```python
from build123d import *

# Parameters (mm, degrees)
HUB_PROFILE_SKETCH_R           = 4.5
HUB_CYLINDER_DEPTH             = 6
ARM_START                      = -4
ARM_DEPTH                      = 3
FLAT_EAR_PROFILE_SKETCH_R      = 0.7
FLAT_MOUNTING_EAR_DEPTH        = 1.6
UPRIGHT_EAR_PROFILE_SKETCH_R   = 0.7
UPRIGHT_MOUNTING_EAR_DEPTH     = 0.8
UPRIGHT_EAR_EXTENSION_SKETCH_W = 1.6
UPRIGHT_EAR_EXTENSION_SKETCH_H = 3.2
UPRIGHT_EAR_EXTENSION_DEPTH    = 0.8
HUB_BORE_CBORE_4_4_D           = 4.4
HUB_BORE_CBORE_4_4_DEPTH       = 100
HUB_BORE_CBORE_4_4_CBORE_D     = 6.4
HUB_BORE_CBORE_4_4_CBORE_DEPTH = 2
ARM_FRAME_CUT_DEPTH            = 18.786996987
ARM_FRAME_CUT_DEPTH_BACK       = 18.786996987
ARM_FRAME_CUT_SKETCH_R         = 0.6
ARM_START_2                    = -1
ARM_WINDOW_CUT_A_DEPTH         = 1
ARM_START_3                    = -3
ARM_WINDOW_CUT_B_DEPTH         = 1


with BuildPart() as part:
    # Hub Profile Sketch → Hub Cylinder (new body)
    with BuildSketch(Plane(origin=(0, 0, 0), x_dir=(1, 0, 0), z_dir=(0, 1, 0))):
        with Locations(Location((0, 0, 0), (0, 0, 270))):
            Circle(HUB_PROFILE_SKETCH_R)
    extrude(amount=HUB_CYLINDER_DEPTH)

    # Arm Profile Sketch → Arm (add)
    with BuildSketch(Plane(origin=(0, 6, 0), x_dir=(1, 0, 0), z_dir=(0, 1, 0)).offset(ARM_START)):
        with BuildLine():
            Line((1.029929577, 4.380553055), (14.486091549, 1.216820293))
            ThreePointArc((14.486091549, 1.216820293), (15.45, 0), (14.486091549, -1.216820293))
            Line((14.486091549, -1.216820293), (1.029929577, -4.380553055))
            ThreePointArc((1.029929577, -4.380553055), (4.5, 0), (1.029929577, 4.380553055))
        make_face()
    extrude(amount=ARM_DEPTH)

    # Flat Ear Profile Sketch → Flat Mounting Ear (add)
    # profile 1 of 2: a face of its own
    with BuildSketch(Plane.XZ):
        with BuildLine():
            Line((-0.677946652, 4.448638931), (-1.807326015, 6.445430372))
            ThreePointArc((-1.807326015, 6.445430372), (-3.987692308, 7.050412049), (-4.592673985, 4.870045756))
            Line((-4.592673985, 4.870045756), (-3.463294622, 2.873254315))
            ThreePointArc((-3.463294622, 2.873254315), (-2.215384615, 3.916895583), (-0.677946652, 4.448638931))
        make_face()
        with Locations(Location((-3.2, 5.657738064, 0), (0, 0, 270))):
            Circle(FLAT_EAR_PROFILE_SKETCH_R, mode=Mode.SUBTRACT)
    # profile 2 of 2: a face of its own
    with BuildSketch(Plane.XZ):
        with BuildLine():
            Line((-0.677946652, -4.448638931), (-1.807326015, -6.445430372))
            ThreePointArc((-1.807326015, -6.445430372), (-3.987692308, -7.050412049), (-4.592673985, -4.870045756))
            Line((-4.592673985, -4.870045756), (-3.463294622, -2.873254315))
            ThreePointArc((-3.463294622, -2.873254315), (-2.215384615, -3.916895583), (-0.677946652, -4.448638931))
        make_face()
        with Locations(Location((-3.2, -5.657738064, 0), (0, 0, 270))):
            Circle(FLAT_EAR_PROFILE_SKETCH_R, mode=Mode.SUBTRACT)
    extrude(amount=-FLAT_MOUNTING_EAR_DEPTH)



with BuildPart() as body_2:
    # Upright Ear Profile Sketch → Upright Mounting Ear (new, symmetric)
    with BuildSketch(Plane.XY):
        with BuildLine():
            Line((-4.5, 6), (-6.5, 6))
            ThreePointArc((-6.5, 6), (-8.1, 4.4), (-6.5, 2.8))
            Line((-6.5, 2.8), (-4.5, 2.8))
            Line((-4.5, 2.8), (-4.5, 6))
        make_face()
        with Locations((-6.5, 4.4)):
            Circle(UPRIGHT_EAR_PROFILE_SKETCH_R, mode=Mode.SUBTRACT)
    extrude(amount=UPRIGHT_MOUNTING_EAR_DEPTH, both=True)


with BuildPart() as part_1:
    add(part.part)

    add(body_2.part)  # Upright Ear Extension merges body 2
    # Upright Ear Extension Sketch → Upright Ear Extension (add, symmetric)
    with BuildSketch(Plane(origin=(-4.5, 0, 0), x_dir=(0, 0, -1), z_dir=(1, 0, 0))):
        with Locations((0, 4.4)):
            Rectangle(UPRIGHT_EAR_EXTENSION_SKETCH_W, UPRIGHT_EAR_EXTENSION_SKETCH_H)
    extrude(amount=UPRIGHT_EAR_EXTENSION_DEPTH, both=True)

    # Hub Bore CBore _4.4
    with Locations(Plane(origin=(0, 6, 0), x_dir=(1, 0, 0), z_dir=(0, 1, 0))):
        with Locations((0, 0)):
            CounterBoreHole(HUB_BORE_CBORE_4_4_D / 2, HUB_BORE_CBORE_4_4_CBORE_D / 2, HUB_BORE_CBORE_4_4_CBORE_DEPTH, depth=HUB_BORE_CBORE_4_4_DEPTH)

    # Arm Frame Cut Sketch → Arm Frame Cut (cut, two sides: drawn at the far end of the back side and taken through both)
    with BuildSketch(Plane(origin=(0, 5, 0), x_dir=(1, 0, 0), z_dir=(0, 1, 0)).offset(-ARM_FRAME_CUT_DEPTH_BACK)):
        with Locations(Location((14.2, 0, 0), (0, 0, 270))):
            Circle(ARM_FRAME_CUT_SKETCH_R)
        with BuildLine():
            Line((12.018798086, 0.769648107), (5.510009379, 2.299955792))
            ThreePointArc((5.510009379, 2.299955792), (5.216619254, 2.20665809), (5.159898403, 1.904061046))
            ThreePointArc((5.159898403, 1.904061046), (5.5, 0), (5.159898403, -1.904061046))
            ThreePointArc((5.159898403, -1.904061046), (5.216619254, -2.20665809), (5.510009379, -2.299955792))
            Line((5.510009379, -2.299955792), (12.018798086, -0.769648107))
            ThreePointArc((12.018798086, -0.769648107), (12.203456694, -0.638324285), (12.243596621, -0.415314119))
            ThreePointArc((12.243596621, -0.415314119), (12.2, 0), (12.243596621, 0.415314119))
            ThreePointArc((12.243596621, 0.415314119), (12.203456694, 0.638324285), (12.018798086, 0.769648107))
        make_face()
    extrude(amount=ARM_FRAME_CUT_DEPTH + ARM_FRAME_CUT_DEPTH_BACK, mode=Mode.SUBTRACT)

    # Arm Window Sketch → Arm Window Cut A (cut)
    with BuildSketch(Plane(origin=(0, 5, 0), x_dir=(1, 0, 0), z_dir=(0, 1, 0)).offset(ARM_START_2)):
        with BuildLine():
            Line((12.96628349, 1.574148524), (4.108268481, 3.656792323))
            ThreePointArc((4.108268481, 3.656792323), (4.716221589, 2.829709158), (5.159898403, 1.904061046))
            ThreePointArc((5.159898403, 1.904061046), (5.216619254, 2.20665809), (5.510009379, 2.299955792))
            Line((5.510009379, 2.299955792), (12.018798086, 0.769648107))
            ThreePointArc((12.018798086, 0.769648107), (12.203456694, 0.638324285), (12.243596621, 0.415314119))
            ThreePointArc((12.243596621, 0.415314119), (12.502961249, 1.058328625), (12.96628349, 1.574148524))
        make_face()
    extrude(amount=ARM_WINDOW_CUT_A_DEPTH, mode=Mode.SUBTRACT)

    # Sketch12_2 → Arm Window Cut B (cut)
    with BuildSketch(Plane(origin=(0, 5, 0), x_dir=(1, 0, 0), z_dir=(0, 1, 0)).offset(ARM_START_3)):
        with BuildLine():
            Line((12.96628349, 1.574148524), (4.108268481, 3.656792323))
            ThreePointArc((4.108268481, 3.656792323), (4.716221589, 2.829709158), (5.159898403, 1.904061046))
            ThreePointArc((5.159898403, 1.904061046), (5.216619254, 2.20665809), (5.510009379, 2.299955792))
            Line((5.510009379, 2.299955792), (12.018798086, 0.769648107))
            ThreePointArc((12.018798086, 0.769648107), (12.203456694, 0.638324285), (12.243596621, 0.415314119))
            ThreePointArc((12.243596621, 0.415314119), (12.502961249, 1.058328625), (12.96628349, 1.574148524))
        make_face()
    extrude(amount=ARM_WINDOW_CUT_B_DEPTH, mode=Mode.SUBTRACT)


solid = part_1.part
```
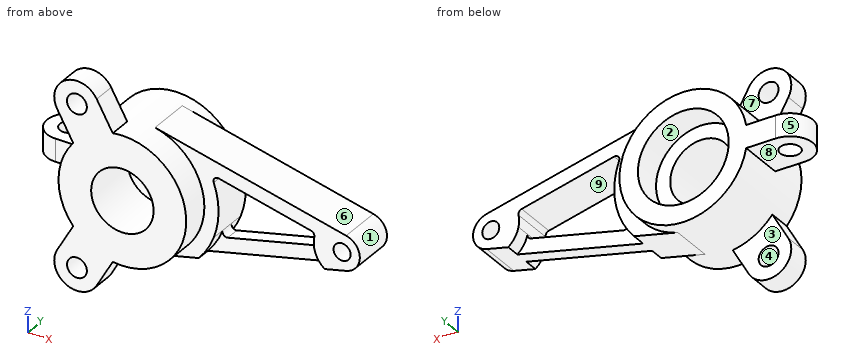
Check sheet for the modelled part. Datum: model origin and axes. Units: mm. Face numbers are marked on the shaded views. A direction names the side the tool comes from. Coordinates: 2 decimals unless noted, no trailing zeros. Order: outer loops, then holes, each group sorted by start corner. A loop starts at its lowest first (then second) coordinate and runs counter-clockwise, first axis right, second up. Notation, with made-up numbers: M -18.5,-22 L 13.5,-22 A34 cw 13.5,13 Z; hole C 16.25,48.25 d3. An arc over 180 degrees is marked long. One line per question, with ' | ' between items. Start each with the question number.
Item 1: Sectioned sample at A-A on z = 0. Record the cut outline in (x, y).
Item 2: Material ranges on line 1 (Z direction, x = 0, y = 5.35); line 2 (Z direction, x = 0, y = 1.3); line 3 (Y direction, x = -3.5, z = -6.5), recorded low to high.
Item 3: Sectioned sample at B-B on y = 4.4. Record the cut outline in (x, z).
Item 4: Sectioned sample at D-D on z = -5.25. Record the cut outline in (x, y), and give its area (3 significant figures).
Item 5: Sectioned sample at C-C on x = 0. Record the cut outline in (y, z), and give its area (3 significant figures).
Item 6: Access from +Z, -Z, +X, -X, +Y, -Y to the whole of each face (thin tool, end or side, straight path). Record for the marked faces 5, 6, 7, 8 and 9.
Item 7: Mould release check, pull along Z, two halves, no side actions. Record for the marked faces 1, 2, 3 and 4: pulls with the +Z half, pulls with the -Z half, needs draft (parallel to the pull), parting line crosses it, or undercut.
Item 8: Gauge pin test, flat ends, axial feed: P1, Ø7, axis at x = 12, z = -1.5, coming from the -Y side; P2, Ø1.5, axis at x = 6, z = -2, coming from the +Y side; P3, Ø2.5, axis at x = 7, z = -2.5, coming from the -Y side. Record the tip position at first contact, or that the pin passes through.
Answer below:
1) outline: M -6.5,2.8 L -4.5,2.8 L -4.5,0 L -2.2,0 L -2.2,4 L -3.2,4 L -3.2,6 L -6.5,6 A1.6 ccw Z; M 2.2,0 L 4.5,0 L 4.5,2 L 5.5,2 L 5.5,5 L 4.5,5 L 4.5,6 L 3.2,6 L 3.2,4 L 2.2,4 Z; M 12.2,2 L 13.6,2 L 13.6,5 L 12.2,5 Z; M 14.8,2 L 15.45,2 L 15.45,5 L 14.8,5 Z; hole C -6.5,4.4 d1.4
2) line 1: z = -4.5 to -3.2, 3.2 to 4.5 | line 2: z = -4.5 to -2.2, 2.2 to 4.5 | line 3: y = 0 to 1.6
3) outline: M -8.1,-0.8 L -7.2,-0.8 L -7.2,0.8 L -8.1,0.8 Z; M -5.8,-0.8 L -4.43,-0.8 A4.5 ccw 1.03,-4.38 L 4.11,-3.66 A5.5 ccw 5.16,1.9 A0.3 cw 5.51,2.3 L 12.02,0.77 A0.3 cw 12.24,0.42 A2 ccw 12.97,-1.57 L 14.49,-1.22 A1.25 ccw 14.49,1.22 L 1.03,4.38 A4.5 ccw -4.43,0.8 L -5.8,0.8 Z; hole C 0,0 d6.4; hole C 14.2,0 d1.2
4) outline: M -4.75,0 L -3.77,0 L -3.77,1.6 L -4.75,1.6 Z; M -2.63,0 L -1.13,0 L -1.13,1.6 L -2.63,1.6 Z | area: 3.96 mm^2
5) outline: M 0,-4.5 L 6,-4.5 L 6,-3.2 L 4,-3.2 L 4,-2.2 L 0,-2.2 Z; M 0,2.2 L 4,2.2 L 4,3.2 L 6,3.2 L 6,4.5 L 0,4.5 Z | area: 23.6 mm^2
6) face 5: +Z, -Z, -X | face 6: +Z, +X, +Y, -Y | face 7: +Z, -X, +Y | face 8: -Z, -X, +Y, -Y | face 9: +Y, -Y
7) face 1: parting line crosses it | face 2: undercut | face 3: needs draft | face 4: undercut
8) P1: stops at y = 2 | P2: stops at y = 4 | P3: stops at y = 3
